```python
from build123d import *

# Parameters (mm, degrees)
SKETCH_1_W             = 84
SKETCH_1_H             = 70
SKETCH_1_R             = 24.25
EXTRUDE_1_DEPTH        = 25
SKETCH_2_W             = 35
SKETCH_2_H             = 9.212728036
CUT_EXTRUDE_1_DEPTH    = 75.087785768
HOLE_WIZARD_M6_1_D     = 5
HOLE_WIZARD_M8_1_D     = 6.8
HOLE_WIZARD_M8_1_DEPTH = 19.75
HOLE_WIZARD_M8_1_TIP   = 2.042926105
CHAMFER_2_SIZE         = 1


with BuildPart() as part:
    # 草图1 → 凸台-拉伸1 (new, symmetric)
    with BuildSketch(Plane.XY):
        Rectangle(SKETCH_1_W, SKETCH_1_H)
        with Locations((0, -9)):
            Circle(SKETCH_1_R, mode=Mode.SUBTRACT)
    extrude(amount=EXTRUDE_1_DEPTH, both=True)

    # 草图2 → 切除-拉伸1 (cut, through all)
    with BuildSketch(Plane.XY.offset(25)):
        with Locations((0, -30.393635982)):
            Rectangle(SKETCH_2_W, SKETCH_2_H)
    extrude(amount=-CUT_EXTRUDE_1_DEPTH, mode=Mode.SUBTRACT)

    # M6 螺纹孔1 (through all)
    with Locations(Plane(origin=(0, 0, -25), x_dir=(-1, 0, 0), z_dir=(0, 0, -1))):
        with Locations((-25.980762114, 6), (25.980762114, 6), (25.980762114, -24), (-25.980762114, -24)):
            Hole(HOLE_WIZARD_M6_1_D / 2)

    # M8 螺纹孔1
    with Locations(Plane(origin=(0, 35, 0), x_dir=(1, 0, 0), z_dir=(0, 1, 0))):
        with Locations((-27.5, 11), (-27.5, -11), (27.5, -11), (27.5, 11), (0, 11), (0, -11)):
            Hole(HOLE_WIZARD_M8_1_D / 2, depth=HOLE_WIZARD_M8_1_DEPTH)
            with Locations((0, 0, -(HOLE_WIZARD_M8_1_DEPTH + HOLE_WIZARD_M8_1_TIP / 2))):  # 118° drill point
                Cone(0, HOLE_WIZARD_M8_1_D / 2, HOLE_WIZARD_M8_1_TIP, mode=Mode.SUBTRACT)

    # 倒角2
    chamfer_2_edges = [part.edges().sort_by_distance(p)[0] for p in [
        (0, 15.25, 25),
        (0, 15.25, -25),
    ]]
    chamfer(chamfer_2_edges, length=CHAMFER_2_SIZE)


solid = part.part
```
Work out the finished part from the listing and answer in its coordinate system (mm). A direction names the side the tool comes from. Coordinates: 2 decimals unless noted, no trailing zeros. Order: outer loops, then holes, each group sorted by start corner. A loop starts at its lowest first (then second) coordinate and runs counter-clockwise, first axis right, second up. Notation, with made-up numbers: (38, 54.25) - (65, 54.25) arc R20 ccw to (65, 87.25) - close; hole circle Ø10 at (58.5, 53). An arc over 180 degrees is marked (long way). Answer as a JSON object with one key per item and string values.
1. A tool of negligible diameter and unlimited length cuts with its end or side. For faces 5 (the face through (-30.64, 24.99, 12.3)), 6 (the face through (-10, 16, -25)), 7 (the face through (17.5, -30, 0)), from which of +Z, -Z, +X, -X, +Y, -Y can it reach the whole face along a straight path? Write none if from no direction.
Output values:
{"face 5": "+Y", "face 6": "-Z, +X, -X, +Y, -Y", "face 7": "+Z, -Z, -Y"}
2. The mould has two halves that part along Y. Classify faces 1 (the face through (25.9, 25, -8)), 2 (the face through (27.32, 8.11, 0.35)), 3 (the face through (25.66, -21.52, 0.35)), 4 (the face through (-1, 35, 0)): +Y half, -Y half, draft (parallel to the pull), parting line (faces both ways), or undercut.
Output values:
{"face 1": "draft", "face 2": "undercut", "face 3": "undercut", "face 4": "+Y half"}
3. Find section C-C on z = -9.5. Count the separate pieces of the cut face and the enclosed holes in it, plus the area to 3 significant figures.
Output values:
{"separate pieces": "2", "enclosed holes": "4", "area": "3,440 mm²"}
4. Each of these flat-tipped pins is pushed along its axis until it touches: P1, Ø10, axis at x = 3, z = -14, coming from the -Y side; P2, Ø4, axis at x = -27.5, z = 11, coming from the +Y side. Where does it stop, or does it pass through?
Output values:
{"P1": "stops at y = 13.89", "P2": "stops at y = 14.41"}
5. Consider line 1 (Z direction, x = -27.5, y = 30.5); line 2 (X direction, y = 21.5, z = -11); line 3 (X direction, y = -25.5, z = 6). Determine where each line is inside the solid, lowest interval first.
Output values:
{"line 1": "z = -25 to -14.4, -7.6 to 7.6, 14.4 to 25", "line 2": "x = -42 to -30.9, -24.1 to -3.4, 3.4 to 24.1, 30.9 to 42", "line 3": "x = -42 to -27.98, -23.98 to -17.77, 17.77 to 23.98, 27.98 to 42"}
6. Find section A-A on y = -9. Determine the outline of the cut face in (x, z).
Output values:
{"outline": "(-42, -25) - (-25.25, -25) - (-24.25, -24) - (-24.25, 24) - (-25.25, 25) - (-42, 25) - close; (24.25, -24) - (25.25, -25) - (42, -25) - (42, 25) - (25.25, 25) - (24.25, 24) - close"}
7. Find section B-B on z = -4. Determine the outline of the cut face in (x, y).
Output values:
{"outline": "(-42, -35) - (-17.5, -35) - (-17.5, -25.79) arc R24.25 cw (long way) to (17.5, -25.79) - (17.5, -35) - (42, -35) - (42, 35) - (-42, 35) - close; hole circle Ø5 at (-25.98, -24); hole circle Ø5 at (-25.98, 6); hole circle Ø5 at (25.98, -24); hole circle Ø5 at (25.98, 6)"}
